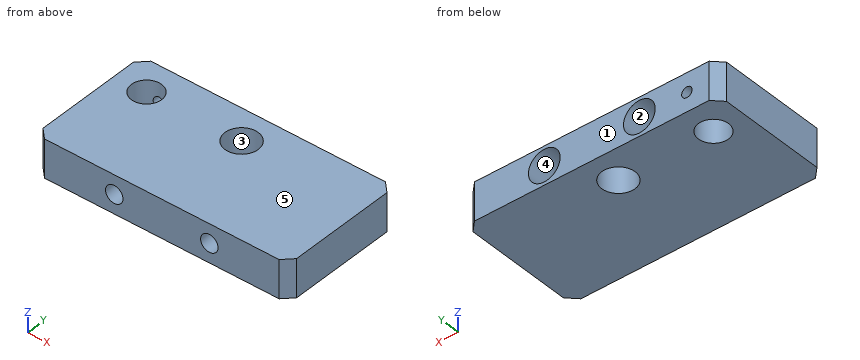
```python
from build123d import *

# Parameters (mm, degrees)
SKETCH1_W                                           = 80
SKETCH1_H                                           = 40
BOSS_EXTRUDE1_DEPTH                                 = 12
SKETCH2_R                                           = 5.25
SKETCH2_R_2                                         = 4.75
CUT_EXTRUDE1_DEPTH                                  = 47.303347611
CBORE_FOR_M5_HEX_SOCKET_HEAD_CAP_SCREW1_D           = 5.5
CBORE_FOR_M5_HEX_SOCKET_HEAD_CAP_SCREW1_CBORE_D     = 10
CBORE_FOR_M5_HEX_SOCKET_HEAD_CAP_SCREW1_CBORE_DEPTH = 35
CHAMFER1_SIZE                                       = 3
M4_TAPPED_HOLE1_D                                   = 3.3
M4_TAPPED_HOLE1_DEPTH                               = 10.1
M4_TAPPED_HOLE1_TIP                                 = 0.991420021


with BuildPart() as part:
    # Sketch1 → Boss-Extrude1 (new body)
    with BuildSketch(Plane.XY):
        Rectangle(SKETCH1_W, SKETCH1_H)
    extrude(amount=BOSS_EXTRUDE1_DEPTH)

    # Sketch2 → Cut-Extrude1 (cut, through all)
    with BuildSketch(Plane.XY.offset(12)):
        with Locations((0, 10)):
            Circle(SKETCH2_R)
        with Locations((-30, 10)):
            Circle(SKETCH2_R_2)
    extrude(amount=-CUT_EXTRUDE1_DEPTH, mode=Mode.SUBTRACT)

    # CBORE for M5 Hex Socket Head Cap Screw1 (through all)
    with Locations(Plane(origin=(0, 20, 0), x_dir=(1, 0, 0), z_dir=(0, 1, 0))):
        with Locations((-15, -6), (15, -6)):
            CounterBoreHole(CBORE_FOR_M5_HEX_SOCKET_HEAD_CAP_SCREW1_D / 2, CBORE_FOR_M5_HEX_SOCKET_HEAD_CAP_SCREW1_CBORE_D / 2, CBORE_FOR_M5_HEX_SOCKET_HEAD_CAP_SCREW1_CBORE_DEPTH)

    # Chamfer1
    chamfer1_edges = [part.edges().sort_by_distance(p)[0] for p in [
        (40, -20, 6),
        (-40, -20, 6),
        (-40, 20, 6),
        (40, 20, 6),
    ]]
    chamfer(chamfer1_edges, length=CHAMFER1_SIZE)

    # M4 Tapped Hole1
    with Locations(Plane(origin=(0, 20, 0), x_dir=(1, 0, 0), z_dir=(0, 1, 0))):
        with Locations((-30, -6)):
            Hole(M4_TAPPED_HOLE1_D / 2, depth=M4_TAPPED_HOLE1_DEPTH)
            with Locations((0, 0, -(M4_TAPPED_HOLE1_DEPTH + M4_TAPPED_HOLE1_TIP / 2))):  # 118° drill point
                Cone(0, M4_TAPPED_HOLE1_D / 2, M4_TAPPED_HOLE1_TIP, mode=Mode.SUBTRACT)


solid = part.part
```
Verification items for the finished model (mm, model axes). Face numbers are marked on the shaded views. A direction names the side the tool comes from. Round coordinates to 2 decimals unless told otherwise and drop trailing zeros. Order: outer loops, then holes, each group sorted by start corner. A loop starts at its lowest first (then second) coordinate and runs counter-clockwise, first axis right, second up. Notation, with made-up numbers: (-16.75, 49.5) - (3.25, 49.5) arc R13 ccw to (3.25, 70.5) - close; hole circle Ø10 at (5.25, 83.5). An arc over 180 degrees is marked (long way). Use CSV: the item, a comma, the result in double quotes. Start each with the question number.
1) Go/stop test with flat-tipped pins: P1, Ø3, axis at x = -12.5, z = 8, coming from the +Y side; P2, Ø4, axis at x = -23, y = 11, coming from the -Z side; P3, Ø3, axis at x = -30, z = 6, coming from the +Y side. Record where each tip stops, or that it passes through.
2) Thickness scan on L1, parallel to Y at x = 0, z = 3.25; L2, parallel to X at y = 9.5, z = 8; L3, parallel to X at y = -4.5, z = 10. Record the ranges inside material, lowest first.
3) Mould release check, pull along Y, two halves, no side actions. Record for the marked faces 1, 2 and 3: +Y half, -Y half, draft (parallel to the pull), parting line (faces both ways), or undercut.
4) Section check B-B, the plane z = 6. State how many separate pieces and enclosed holes the cut face has, plus the area to 3 significant figures.
5) Section check C-C, the plane x = 15. Record the cut outline in (y, z), plus the area to 4 significant figures.
6) Access from +Z, -Z, +X, -X, +Y, -Y to the whole of each face (thin tool, end or side, straight path). Record for the marked faces 4 and 5.
7) Section check A-A, the plane y = 10. Record the cut outline in (x, z).
8) Section check D-D, the plane x = -30. Record the cut outline in (y, z), plus the area to 3 significant figures.
Answers:
1,P1,"stops at y = -15"
1,P2,"stops at z = 0"
1,P3,"stops at y = 5.49"
2,L1,"y = -20 to 4.75, 15.25 to 20"
2,L2,"x = -40 to -34.72, -25.28 to -19.58, -10.42 to -5.23, 5.23 to 10.42, 19.58 to 40"
2,L3,"x = -40 to -18, -12 to 12, 18 to 40"
3,face 1,"+Y half"
3,face 2,"draft"
3,face 3,"undercut"
4,separate pieces,"3"
4,enclosed holes,"1"
4,area,"2,250 mm²"
5,outline,"(-20, 0) - (20, 0) - (20, 1) - (-15, 1) - (-15, 3.25) - (-20, 3.25) - close; (-20, 8.75) - (-15, 8.75) - (-15, 11) - (20, 11) - (20, 12) - (-20, 12) - close"
5,area,"102.5 mm²"
6,face 4,"+Y"
6,face 5,"+Z, +X, -X, +Y, -Y"
7,outline,"(-40, 0) - (-34.75, 0) - (-34.75, 12) - (-40, 12) - close; (-25.25, 0) - (-5.25, 0) - (-5.25, 12) - (-25.25, 12) - close; (5.25, 0) - (40, 0) - (40, 12) - (5.25, 12) - close; hole circle Ø10 at (-15, 6); hole circle Ø10 at (15, 6)"
8,outline,"(-20, 0) - (5.25, 0) - (5.25, 12) - (-20, 12) - close; (14.75, 0) - (20, 0) - (20, 4.35) - (14.75, 4.35) - close; (14.75, 7.65) - (20, 7.65) - (20, 12) - (14.75, 12) - close"
8,area,"349 mm²"
